from build123d import *

# Parameters (mm, degrees)
SKETCH1_R           = 50
BOSS_EXTRUDE1_DEPTH = 26
SKETCH2_R           = 66.5
BOSS_EXTRUDE2_DEPTH = 216
SKETCH3_R           = 50
BOSS_EXTRUDE3_DEPTH = 26
SKETCH4_R           = 40
CUT_EXTRUDE1_DEPTH  = 79
CUT_EXTRUDE2_START  = -79
SKETCH5_R           = 40
CUT_EXTRUDE2_DEPTH  = 79
SKETCH6_R           = 36.5
CUT_EXTRUDE3_DEPTH  = 212.1054239
CHAMFER1_SIZE       = 10
CHAMFER2_SIZE       = 10


with BuildPart() as part:
    # Sketch1 → Boss-Extrude1 (new body)
    with BuildSketch(Plane.XY):
        with Locations(Location((0, 0, 0), (0, 0, 180))):
            Circle(SKETCH1_R)
    extrude(amount=BOSS_EXTRUDE1_DEPTH)

    # Sketch2 → Boss-Extrude2 (add)
    with BuildSketch(Plane.XY.offset(26)):
        Circle(SKETCH2_R)
    extrude(amount=BOSS_EXTRUDE2_DEPTH)

    # Sketch3 → Boss-Extrude3 (add)
    with BuildSketch(Plane.XY.offset(242)):
        with Locations(Location((0, 0, 0), (0, 0, 180))):
            Circle(SKETCH3_R)
    extrude(amount=BOSS_EXTRUDE3_DEPTH)

    # Sketch4 → Cut-Extrude1 (cut)
    with BuildSketch(Plane.XY.offset(268)):
        Circle(SKETCH4_R)
    extrude(amount=-CUT_EXTRUDE1_DEPTH, mode=Mode.SUBTRACT)

    # Sketch5 → Cut-Extrude2 (cut)
    with BuildSketch(Plane(origin=(0, 0, 0), x_dir=(-1, 0, 0), z_dir=(0, 0, -1)).offset(CUT_EXTRUDE2_START)):
        with Locations(Location((0, 0, 0), (0, 0, 180))):
            Circle(SKETCH5_R)
    extrude(amount=CUT_EXTRUDE2_DEPTH, mode=Mode.SUBTRACT)

    # Sketch6 → Cut-Extrude3 (cut, through all)
    with BuildSketch(Plane(origin=(0, 0, 79), x_dir=(-1, 0, 0), z_dir=(0, 0, -1))):
        Circle(SKETCH6_R)
    extrude(amount=-CUT_EXTRUDE3_DEPTH, mode=Mode.SUBTRACT)

    # Chamfer1
    chamfer1_edges = [part.edges().sort_by_distance(p)[0] for p in [
        (-66.5, 0, 242),
    ]]
    chamfer(chamfer1_edges, length=CHAMFER1_SIZE)

    # Chamfer2
    chamfer2_edges = [part.edges().sort_by_distance(p)[0] for p in [
        (-66.5, 0, 26),
    ]]
    chamfer(chamfer2_edges, length=CHAMFER2_SIZE)


solid = part.part
Geometry: final body of the model. Coordinates: model frame, mm. A direction names the side the tool comes from. Give positions to 0.01 mm unless a question says otherwise; leave off trailing zeros. Write each loop counter-clockwise with the first axis right and the second up, starting at its lowest first coordinate (ties: lowest second). Pieces come first, ordered by that corner, then holes.
(1) Cut plane A-A, the plane y = 0. Return loops of the section in (x, z), then the cut area to 3 significant figures.
(2) Access query for faces 1 (the cylindrical face through (35.75, 56.073, 132.628)), 2 (the cylindrical face through (-8.67, -39.05, 229.05)), 3 (the cylindrical face through (-47.69, -15.02, 12.82)). Directions: +Z, -Z, +X, -X, +Y, -Y. A direction counts if a zero-diameter tool reaches every point of the face in a straight line with its end or side. Return the directions, or none.
(3) Cut plane C-C, the plane z = 114. Return loops of the section in (x, y), then the cut area to 3 significant figures.
(4) First-contact query: P1, Ø8, axis at x = -17.5, z = 187, coming from the -Y side; P2, Ø10, axis at y = -37, z = 165, coming from the -X side; P3, Ø1, axis at y = -40, z = 56, coming from the +X side. Flat tips, straight axial feed; report the tip coordinate or a pass-through.
(5) Cut plane D-D, the plane z = 199. Return loops of the section in (x, y).
(6) Ray query, line 1 (Y direction, x = 0, z = 163); line 2 (Y direction, x = 0, z = 219.5); line 3 (Z direction, x = -48, y = -23.5). Return the intervals inside material, ascending.
(7) Mould query, pull axis Y, two halves, no side actions, for faces 4 (the cylindrical face through (7.912, -35.632, 133.23)), 5 (the cylindrical face through (-39.96, -1.76, 40.05)), 6 (the conical face through (-45.222, -34.675, 241.514)), 7 (the flat face through (22, -34, 268)). Classes: released by +Y, released by -Y, zero draft, split by the parting line, or undercut.
Values follow:
1. outline: (-66.5, 36) - (-56.5, 26) - (-50, 26) - (-50, 0) - (-40, 0) - (-40, 79) - (-36.5, 79) - (-36.5, 189) - (-40, 189) - (-40, 268) - (-50, 268) - (-50, 242) - (-56.5, 242) - (-66.5, 232) - close; (36.5, 79) - (40, 79) - (40, 0) - (50, 0) - (50, 26) - (56.5, 26) - (66.5, 36) - (66.5, 232) - (56.5, 242) - (50, 242) - (50, 268) - (40, 268) - (40, 189) - (36.5, 189) - close
1. area: 13,100 mm2
2. face 1: +Z, -Z
2. face 2: +Z
2. face 3: -Z
3. outline: circle Ø133 at (0, 0); hole circle Ø73 at (0, 0)
3. area: 9,710 mm2
4. P1: stops at y = -65.12
4. P2: stops at x = -58.29
4. P3: stops at x = 53.5
5. outline: circle Ø133 at (0, 0); hole circle Ø80 at (0, 0)
6. line 1: y = -66.5 to -36.5, 36.5 to 66.5
6. line 2: y = -66.5 to -40, 40 to 66.5
6. line 3: z = 26 to 242
7. face 4: undercut
7. face 5: undercut
7. face 6: split by the parting line
7. face 7: zero draft
